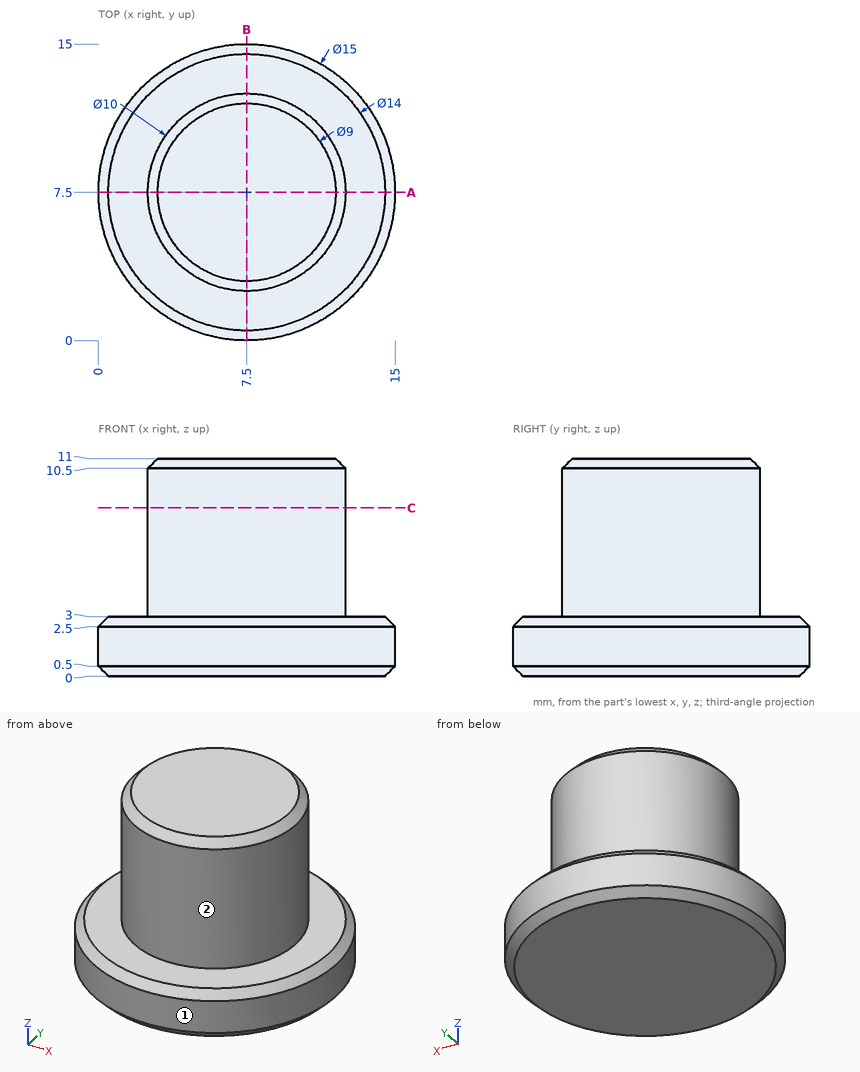
Verification items for this drawing (mm, ordinates from the low corner). A direction names the side the tool comes from. Give positions to 0.01 mm unless a question says otherwise; leave off trailing zeros. Loops run counter-clockwise (first coordinate to the right, second up) from the corner with the lowest first, then second, coordinate; pieces in that order, holes last. Notation, with made-up numbers: M 70,74.25 L 115,74.25 A29 cw 115,100.25 Z; hole C -29.75,-19 d4. An arc over 180 degrees is marked long. Answer as CSV lines item,"result".
Item 1: Access from +Z, -Z, +X, -X, +Y, -Y to the whole of each face (thin tool, end or side, straight path). Record for the marked faces 1 and 2.
Values:
face 1,"+Z, -Z"
face 2,"+Z"
Item 2: Cross-section at A-A on y = 7.5. Record the cut outline in (x, z).
Values:
outline,"M 0,0.5 L 0.5,0 L 14.5,0 L 15,0.5 L 15,2.5 L 14.5,3 L 12.5,3 L 12.5,10.5 L 12,11 L 3,11 L 2.5,10.5 L 2.5,3 L 0.5,3 L 0,2.5 Z"
Item 3: Depth check by flat-ended pin: P1, Ø3, axis at y = 13.5, z = 7, coming from the -X side; P2, Ø2, axis at y = 3.5, z = 6, coming from the -X side; P3, Ø2, axis at y = 5.5, z = 6, coming from the -X side. Enter the tip coordinate at first touch or a pass-through.
Values:
P1,"stops at x = 5.32"
P2,"stops at x = 3.5"
P3,"stops at x = 2.6"
Item 4: Material ranges on line 1 (Z direction, x = 13, y = 5.5); line 2 (Y direction, x = 6, z = 10.75); line 3 (Y direction, x = 12, z = 6), recorded low to high.
Values:
line 1,"z = 0 to 3"
line 2,"y = 2.99 to 12.01"
line 3,"y = 5.32 to 9.68"
Item 5: Cross-section at C-C on z = 8.5. Record the cut outline in (x, y).
Values:
outline,"C 7.5,7.5 d10"
